from build123d import *

# Parameters (mm, degrees)
SKETCH_1_3_W        = 28
SKETCH_1_3_H        = 28
BOSS_EXTRUDE1_DEPTH = 1
SKETCH_1_3_2_W      = 30
SKETCH_1_3_2_H      = 30
SKETCH_1_3_2_W_2    = 28
SKETCH_1_3_2_H_2    = 28
EXTRUDE_THIN1_DEPTH = 5
SKETCH2_R           = 11
CUT_EXTRUDE1_DEPTH  = 5


with BuildPart() as part:
    # Sketch 1_3 → Boss-Extrude1 (new body)
    with BuildSketch(Plane.XY):
        Rectangle(SKETCH_1_3_W, SKETCH_1_3_H)
    extrude(amount=BOSS_EXTRUDE1_DEPTH)

    # Sketch 1_3 2 → Extrude-Thin1 (add)
    with BuildSketch(Plane.XY):
        Rectangle(SKETCH_1_3_2_W, SKETCH_1_3_2_H)
        Rectangle(SKETCH_1_3_2_W_2, SKETCH_1_3_2_H_2, mode=Mode.SUBTRACT)
    extrude(amount=EXTRUDE_THIN1_DEPTH)

    # Sketch2 → Cut-Extrude1 (cut)
    with BuildSketch(Plane.XY.offset(1)):
        Circle(SKETCH2_R)
    extrude(amount=-CUT_EXTRUDE1_DEPTH, mode=Mode.SUBTRACT)


solid = part.part
Geometry check sheet. Reference: the model listing, model coordinates, mm. A direction names the side the tool comes from. Round coordinates to 2 decimals unless told otherwise and drop trailing zeros. Loops run counter-clockwise (first coordinate to the right, second up) from the corner with the lowest first, then second, coordinate; pieces in that order, holes last.
Item 1: Mould release check, pull along X, two halves, no side actions. Record for faces 3 (the flat face through (14, 0, 3)), 4 (the flat face through (-14, 0, 3)), 5 (the flat face through (-1.2, -14.4, 5)), 6 (the flat face through (-15, 0, 2)): pulls with the +X half, pulls with the -X half, needs draft (parallel to the pull), parting line crosses it, or undercut.
Item 2: Cross-section at A-A on y = 0. Record the boundary of the cut face in (x, z), then the cut area to 3 significant figures.
Item 3: Gauge pin test, flat end, axial feed: pin 1 (2 mm diameter, centred on x = -9.5, y = -7.5, fed in from +Z). Record the tip position at first contact, or that the pin passes through.
Item 4: Access from +Z, -Z, +X, -X, +Y, -Y to the whole of each face (thin tool, end or side, straight path). Record for faces 1 (the flat face through (0, -14, 3)), 2 (the flat face through (0, -15, 2)).
Item 5: Cross-section at C-C on z = 1.4. Record the boundary of the cut face in (x, y).
Item 6: Cross-section at D-D on y = -12.25. Record the boundary of the cut face in (x, z).
Item 7: Thickness scan on line 1 (Y direction, x = -11.75, z = 2.55); line 2 (Y direction, x = 0, z = 0.75). Record the ranges inside material, lowest first.
Answer sheet:
1. face 3: undercut
1. face 4: undercut
1. face 5: needs draft
1. face 6: pulls with the -X half
2. outline: (-15, 0) - (-11, 0) - (-11, 1) - (-14, 1) - (-14, 5) - (-15, 5) - close; (11, 0) - (15, 0) - (15, 5) - (14, 5) - (14, 1) - (11, 1) - close
2. area: 16.0 mm2
3. pin 1: stops at z = 1
4. face 1: +Z
4. face 2: +Z, -Z, +X, -X, -Y
5. outline: (-15, -15) - (15, -15) - (15, 15) - (-15, 15) - close; hole (-14, -14) - (14, -14) - (14, 14) - (-14, 14) - close
6. outline: (-15, 0) - (15, 0) - (15, 5) - (14, 5) - (14, 1) - (-14, 1) - (-14, 5) - (-15, 5) - close
7. line 1: y = -15 to -14, 14 to 15
7. line 2: y = -15 to -11, 11 to 15
